Geometry: final body of the model. Coordinates: model frame, mm. A direction names the side the tool comes from. Coordinates: 2 decimals unless noted, no trailing zeros. Write each loop counter-clockwise with the first axis right and the second up, starting at its lowest first coordinate (ties: lowest second). Pieces come first, ordered by that corner, then holes. Notation, with made-up numbers: (2.25, -14) - (58.25, -14) arc R32 cw to (58.25, 12) - close; hole circle Ø8 at (-27.75, 10.25). An arc over 180 degrees is marked (long way). Put each result on its own line as item: value.
```python
from build123d import *

# Parameters (mm, degrees)
SKETCH1_W     = 26
SKETCH1_H     = 10
CHAMFER1_SIZE = 2


with BuildPart() as part:
    # Sketch1 → Revolve1 (revolve)
    with BuildSketch(Plane(origin=(0, 0, 0), x_dir=(0, 0, -1), z_dir=(1, 0, 0)), mode=Mode.PRIVATE) as revolve1_sk:
        with Locations((13, 40)):
            Rectangle(SKETCH1_W, SKETCH1_H)
        Polygon((26, 45), (26, 35), (36, 35), (36, 46), (26, 46), align=None)
    revolve(revolve1_sk.sketch.rotate(Axis((0, 0, 0), (0, 0, -1)), 90), axis=Axis((0, 0, 0), (0, 0, -1)))

    # Chamfer1
    chamfer1_edges = [part.edges().sort_by_distance(p)[0] for p in [
        (-45, 0, 0),
        (-46, 0, -36),
        (-35, 0, -36),
        (-35, 0, 0),
    ]]
    chamfer(chamfer1_edges, length=CHAMFER1_SIZE)


solid = part.part
```
1. Set-up query: faces 1 (the cylindrical face through (20.765, 39.923, -14.168)), 2 (the cylindrical face through (-7.587, 34.168, -18.224)). Return all of +Z, -Z, +X, -X, +Y, -Y with unobstructed straight access to the full face (end or side cutting, diameter ignored); none if empty.
Answer below:
face 1: +Z
face 2: +Z, -Z
2. Section query A-A (x = 0). Return loops of the section in (y, z), then the cut area to 3 significant figures.
Answer below:
outline: (-46, -34) - (-44, -36) - (-37, -36) - (-35, -34) - (-35, -2) - (-37, 0) - (-43, 0) - (-45, -2) - (-45, -26) - (-46, -26) - close; (35, -34) - (37, -36) - (44, -36) - (46, -34) - (46, -26) - (45, -26) - (45, -2) - (43, 0) - (37, 0) - (35, -2) - close
area: 724 mm²
3. Section query D-D (z = -29.5). Return loops of the section in (x, y).
Answer below:
outline: circle Ø92 at (0, 0); hole circle Ø70 at (0, 0)
4. Pin query (flat end, axial travel): pin 1 Ø4 at (y, z) = (36, -7.5) entering from -X; pin 2 Ø2 at (x, z) = (1.5, -28.5) entering from -Y; pin 3 Ø4 at (x, z) = (-9, -16) entering from +Y. Return the tip coordinate at first contact, or that it passes through.
Answer below:
pin 1: stops at x = -29.48
pin 2: stops at y = -46
pin 3: stops at y = 44.45
5. Ray query, probe 1 along Y at (x, z) = (0, -17); probe 2 along Y at (x, z) = (-1, -30.5); probe 3 along X at (y, z) = (24.5, -8.5) (3 decimals). Return the intervals inside material, ascending. Write a range as from..to.
Answer below:
probe 1: y = -45..-35, 35..45
probe 2: y = -45.99..-34.99, 34.99..45.99
probe 3: x = -37.746..-24.995, 24.995..37.746
6. Mould query, pull axis X, two halves, no side actions, for faces 3 (the conical face through (33.503, -10.551, -34.125)), 4 (the conical face through (41.134, -12.954, -0.125)), 5 (the flat face through (34, 30, -26)). Classes: +X half, -X half, draft (parallel to the pull), parting line (faces both ways), or undercut.
Answer below:
face 3: undercut
face 4: parting line
face 5: draft
7. Section query C-C (z = -12). Return loops of the section in (x, y), then the cut area to 3 significant figures.
Answer below:
outline: circle Ø90 at (0, 0); hole circle Ø70 at (0, 0)
area: 2,510 mm²
